Geometry: final body of the model. Coordinates: model frame, mm. Face numbers are marked on the shaded views. A direction names the side the tool comes from. Give positions to 0.01 mm unless a question says otherwise; leave off trailing zeros. Write each loop counter-clockwise with the first axis right and the second up, starting at its lowest first coordinate (ties: lowest second). Pieces come first, ordered by that corner, then holes. Notation, with made-up numbers: (77.25, -14) -> (119.25, -14) arc R8 cw to (119.25, 0) -> close; hole circle Ø6 at (52.25, 47.25). An arc over 180 degrees is marked (long way). Answer in a Markdown table with one row per item. Add a question column.
Item 1: Access query for the marked faces 1 and 2. Directions: +Z, -Z, +X, -X, +Y, -Y. A direction counts if a zero-diameter tool reaches every point of the face in a straight line with its end or side. Return the directions, or none.
Item 2: Section query B-B on x = 61. Output: boundary loops of the cut face in (y, z).
Item 3: First-contact query: P1, Ø1, axis at y = 148, z = 331, coming from the -X side; P2, Ø2, axis at y = 24.5, z = 16, coming from the +X side; P3, Ø8, axis at y = 98.5, z = -342, coming from the +X side; P4, Ø12, axis at y = 36.5, z = -257.5, coming from the +X side. Flat tips, straight axial feed; report the tip coordinate or a pass-through.
Item 4: Material intervals for probe 1 along X at (y, z) = (74, 122); probe 2 along X at (y, z) = (17.5, 419), sorted ascending. Write a range as from..to.
Item 5: Section query A-A on z = -293. Output: boundary loops of the cut face in (x, y), plus the area to 3 significant figures.
```python
from build123d import *

# Parameters (mm, degrees)
BOSS_EXTRUDE1_DEPTH = 457.2


with BuildPart() as part:
    # Sketch1 → Boss-Extrude1 (new, symmetric)
    with BuildSketch(Plane.XY):
        with BuildLine():
            Line((0, 200), (0, 0))
            Line((0, 0), (200, 0))
            Line((200, 0), (200, 9.333333333))
            ThreePointArc((200, 9.333333333), (198.633164979, 12.633164979), (195.333333333, 14))
            Line((195.333333333, 14), (32, 14))
            ThreePointArc((32, 14), (19.272077939, 19.272077939), (14, 32))
            Line((14, 32), (14, 195.333333333))
            ThreePointArc((14, 195.333333333), (12.633164979, 198.633164979), (9.333333333, 200))
            Line((9.333333333, 200), (0, 200))
        make_face()
    extrude(amount=BOSS_EXTRUDE1_DEPTH, both=True)


solid = part.part
```
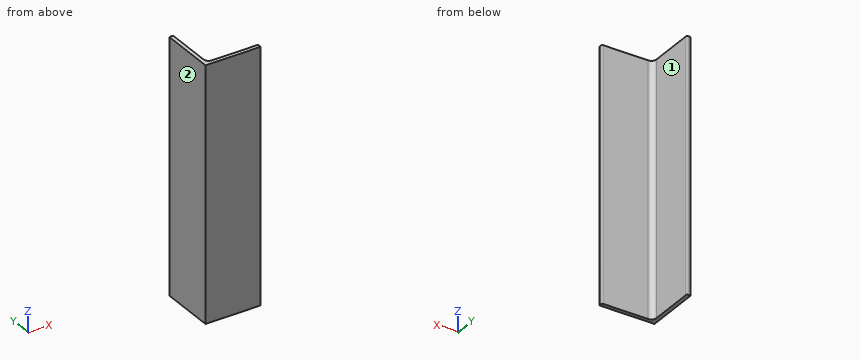
Findings below:
| question | item | result |
|---|---|---|
| 1 | face 1 | +Z, -Z, +X, +Y |
| 1 | face 2 | +Z, -Z, -X, +Y, -Y |
| 2 | outline | (0, -457.2) -> (14, -457.2) -> (14, 457.2) -> (0, 457.2) -> close |
| 3 | P1 | stops at x = 0 |
| 3 | P2 | stops at x = 16.13 |
| 3 | P3 | stops at x = 14 |
| 3 | P4 | stops at x = 14.06 |
| 4 | probe 1 | x = 0..14 |
| 4 | probe 2 | x = 0..21.33 |
| 5 | outline | (0, 0) -> (200, 0) -> (200, 9.33) arc R4.67 ccw to (195.33, 14) -> (32, 14) arc R18 cw to (14, 32) -> (14, 195.33) arc R4.67 ccw to (9.33, 200) -> (0, 200) -> close |
| 5 | area | 5,460 mm^2 |
